Read the model definition and answer for the solid it produces. Units are mm, in the model's axes. Give positions to 0.01 mm unless a question says otherwise; leave off trailing zeros. Loops run counter-clockwise (first coordinate to the right, second up) from the corner with the lowest first, then second, coordinate; pieces in that order, holes last. Notation, with made-up numbers: (46, 85.5) -> (54, 85.5) arc R26 ccw to (54, 103.5) -> close; hole circle Ø5 at (-30, -1). An arc over 180 degrees is marked (long way). Return JSON: item names as keys, results as strings. Group by question number.
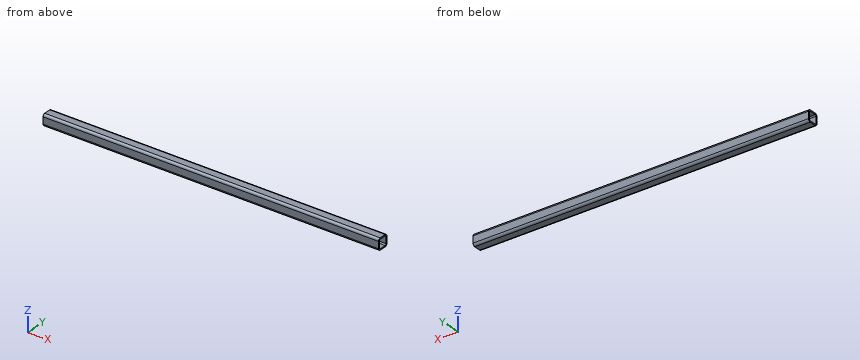
from build123d import *

# Parameters (mm, degrees)
SQUARE_TUBE_40_X_40_X_4_1_DEPTH = 1192


with BuildPart() as part:
    # Sketch1 → Square Tube 40 X 40 X 4(1) (new body)
    with BuildSketch(Plane.YZ.offset(-1000)):
        with BuildLine():
            Line((-12, -20), (12, -20))
            ThreePointArc((12, -20), (17.656854249, -17.656854249), (20, -12))
            Line((20, -12), (20, 12))
            ThreePointArc((20, 12), (17.656854249, 17.656854249), (12, 20))
            Line((12, 20), (-12, 20))
            ThreePointArc((-12, 20), (-17.656854249, 17.656854249), (-20, 12))
            Line((-20, 12), (-20, -12))
            ThreePointArc((-20, -12), (-17.656854249, -17.656854249), (-12, -20))
        make_face()
        with BuildLine():
            Line((-12, -16), (12, -16))
            ThreePointArc((12, -16), (14.828427125, -14.828427125), (16, -12))
            Line((16, -12), (16, 12))
            ThreePointArc((16, 12), (14.828427125, 14.828427125), (12, 16))
            Line((12, 16), (-12, 16))
            ThreePointArc((-12, 16), (-14.828427125, 14.828427125), (-16, 12))
            Line((-16, 12), (-16, -12))
            ThreePointArc((-16, -12), (-14.828427125, -14.828427125), (-12, -16))
        make_face(mode=Mode.SUBTRACT)
    extrude(amount=SQUARE_TUBE_40_X_40_X_4_1_DEPTH)


solid = part.part
1. Section A-A on y = 3 is taken. Determine the outline of the cut face in (x, z).
2. Straight lines are drawn through the part: line 1 (Z direction, x = -577, y = -9); line 2 (Y direction, x = -434, z = 13). For each, find the intervals that lie inside material, in ascending order. Write a range as from..to.
3. Flat-ended cylindrical pins translate along their axes: pin 1 Ø12 at (x, z) = (-879, 15.5) entering from -Y; pin 2 Ø3 at (y, z) = (13.5, 6.5) entering from +X; pin 3 Ø5 at (x, y) = (31, -15.5) entering from +Z; pin 4 Ø1.5 at (x, y) = (-45.5, -14.5) entering from -Z. Find the tip coordinate at first contact, or state that the pin passes through.
4. Section C-C on x = -672 is taken. Determine the outline of the cut face in (y, z).
Completed:
{
 "1": {"outline": "(-1000, -20) -> (192, -20) -> (192, -16) -> (-1000, -16) -> close; (-1000, 16) -> (192, 16) -> (192, 20) -> (-1000, 20) -> close"},
 "2": {"line 1": "z = -20..-16, 16..20", "line 2": "y = -19.94..-15.87, 15.87..19.94"},
 "3": {"pin 1": "stops at y = -20", "pin 2": "passes through", "pin 3": "stops at z = 19.94", "pin 4": "stops at z = -19.81"},
 "4": {"outline": "(-20, -12) arc R8 ccw to (-12, -20) -> (12, -20) arc R8 ccw to (20, -12) -> (20, 12) arc R8 ccw to (12, 20) -> (-12, 20) arc R8 ccw to (-20, 12) -> close; hole (-16, -12) arc R4 ccw to (-12, -16) -> (12, -16) arc R4 ccw to (16, -12) -> (16, 12) arc R4 ccw to (12, 16) -> (-12, 16) arc R4 ccw to (-16, 12) -> close"}
}
